Check sheet for the modelled part. Datum: model origin and axes. Units: mm. Face numbers are marked on the shaded views. Give positions to 0.01 mm unless a question says otherwise; leave off trailing zeros. Write each loop counter-clockwise with the first axis right and the second up, starting at its lowest first coordinate (ties: lowest second). Pieces come first, ordered by that corner, then holes. Notation, with made-up numbers: (59, 35) -> (116, 35) arc R19 ccw to (116, 44) -> close; hole circle Ø3 at (-6.75, 17). An arc over 180 degrees is marked (long way). Write each question's results on one line, items separated by ' | '. Start each with the question number.
```python
from build123d import *

# Parameters (mm, degrees)
SKETCH1_R           = 25
BOSS_EXTRUDE1_DEPTH = 3
CHAMFER1_SIZE       = 1
SKETCH2_R           = 2.75
CUT_EXTRUDE1_DEPTH  = 3


with BuildPart() as part:
    # Sketch1 → Boss-Extrude1 (new body)
    with BuildSketch(Plane.XY):
        Circle(SKETCH1_R)
    extrude(amount=BOSS_EXTRUDE1_DEPTH)

    # Chamfer1
    chamfer1_edges = [part.edges().sort_by_distance(p)[0] for p in [
        (-25, 0, 3),
    ]]
    chamfer(chamfer1_edges, length=CHAMFER1_SIZE)

    # Sketch2 → Cut-Extrude1 (cut)
    with BuildSketch(Plane.XY.offset(3)):
        with Locations((20, 0)):
            Circle(SKETCH2_R)
        with Locations((0, -20)):
            Circle(SKETCH2_R)
        with Locations((-20, 0)):
            Circle(SKETCH2_R)
        with Locations((0, 20)):
            Circle(SKETCH2_R)
    extrude(amount=-CUT_EXTRUDE1_DEPTH, mode=Mode.SUBTRACT)


solid = part.part
```
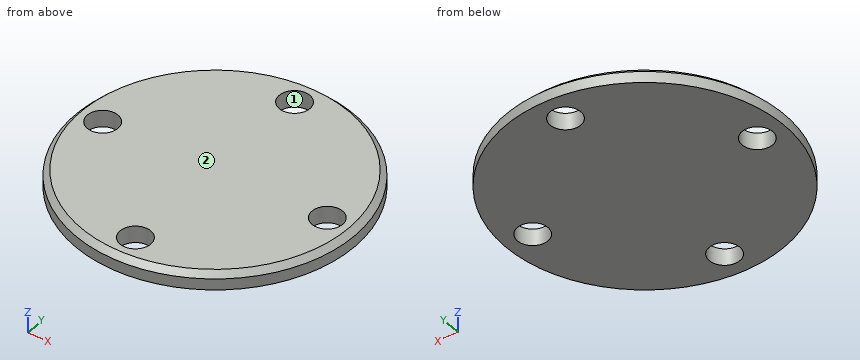
Item 1: Thickness scan on probe 1 along Y at (x, z) = (0, 1.65); probe 2 along X at (y, z) = (-1.5, 0.35); probe 3 along Z at (x, y) = (14, 19.5). Record the ranges inside material, lowest first. Write a range as from..to.
Item 2: Section check C-C on z = 1.4. Record the boundary of the cut face in (x, y).
Item 3: Mould release check, pull along Y, two halves, no side actions. Record for the marked faces 1 and 2: pulls with the +Y half, pulls with the -Y half, needs draft (parallel to the pull), parting line crosses it, or undercut.
Item 4: Depth check by flat-ended pin: pin 1 Ø4.5 at (x, y) = (0, 20) entering from +Z. Enter the tip coordinate at first touch or a pass-through.
Item 5: Section check A-A on x = 0. Record the boundary of the cut face in (y, z).
Check sheet entries:
1) probe 1: y = -25..-22.75, -17.25..17.25, 22.75..25 | probe 2: x = -24.95..-22.3, -17.7..17.7, 22.3..24.95 | probe 3: z = 0..2.99
2) outline: circle Ø50 at (0, 0); hole circle Ø5.5 at (-20, 0); hole circle Ø5.5 at (0, -20); hole circle Ø5.5 at (0, 20); hole circle Ø5.5 at (20, 0)
3) face 1: undercut | face 2: needs draft
4) pin 1: passes through
5) outline: (-25, 0) -> (-22.75, 0) -> (-22.75, 3) -> (-24, 3) -> (-25, 2) -> close; (-17.25, 0) -> (17.25, 0) -> (17.25, 3) -> (-17.25, 3) -> close; (22.75, 0) -> (25, 0) -> (25, 2) -> (24, 3) -> (22.75, 3) -> close
